```python
from build123d import *

# Parameters (mm, degrees)
SKETCH1_R             = 15
BOSS_EXTRUDE1_DEPTH   = 1075
SKETCH2_R             = 11
BOSS_EXTRUDE2_DEPTH   = 10
BOSS_EXTRUDE3_START   = 10
SKETCH3_R             = 11
BOSS_EXTRUDE3_DEPTH   = 10
M8_TAPPED_HOLE1_D     = 6.8
M8_TAPPED_HOLE1_DEPTH = 19.75
M8_TAPPED_HOLE1_TIP   = 2.042926105
M8_TAPPED_HOLE2_D     = 6.8
M8_TAPPED_HOLE2_DEPTH = 19.75
M8_TAPPED_HOLE2_TIP   = 2.042926105


with BuildPart() as part:
    # Sketch1 → Boss-Extrude1 (new body)
    with BuildSketch(Plane(origin=(0, 0, 0), x_dir=(1, 0, 0), z_dir=(0, 1, 0))):
        with Locations(Location((0, 0, 0), (0, 0, 270))):
            Circle(SKETCH1_R)
    extrude(amount=BOSS_EXTRUDE1_DEPTH)

    # Sketch2 → Boss-Extrude2 (add)
    with BuildSketch(Plane(origin=(0, 1075, 0), x_dir=(1, 0, 0), z_dir=(0, 1, 0))):
        with Locations(Location((0, 0, 0), (0, 0, 270))):
            Circle(SKETCH2_R)
    extrude(amount=BOSS_EXTRUDE2_DEPTH)

    # Sketch3 → Boss-Extrude3 (add)
    with BuildSketch(Plane.XZ.offset(BOSS_EXTRUDE3_START)):
        with Locations(Location((0, 0, 0), (0, 0, 90))):
            Circle(SKETCH3_R)
    extrude(amount=-BOSS_EXTRUDE3_DEPTH)

    # M8 Tapped Hole1
    with Locations(Plane(origin=(0, -10, 0), x_dir=(-1, 0, 0), z_dir=(0, -1, 0))):
        with Locations((0, 0)):
            Hole(M8_TAPPED_HOLE1_D / 2, depth=M8_TAPPED_HOLE1_DEPTH)
            with Locations((0, 0, -(M8_TAPPED_HOLE1_DEPTH + M8_TAPPED_HOLE1_TIP / 2))):  # 118° drill point
                Cone(0, M8_TAPPED_HOLE1_D / 2, M8_TAPPED_HOLE1_TIP, mode=Mode.SUBTRACT)

    # M8 Tapped Hole2
    with Locations(Plane(origin=(0, 1085, 0), x_dir=(1, 0, 0), z_dir=(0, 1, 0))):
        with Locations((0, 0)):
            Hole(M8_TAPPED_HOLE2_D / 2, depth=M8_TAPPED_HOLE2_DEPTH)
            with Locations((0, 0, -(M8_TAPPED_HOLE2_DEPTH + M8_TAPPED_HOLE2_TIP / 2))):  # 118° drill point
                Cone(0, M8_TAPPED_HOLE2_D / 2, M8_TAPPED_HOLE2_TIP, mode=Mode.SUBTRACT)


solid = part.part
```
Build history of the part. All positions in model axes, mm. A direction names the side the tool comes from. Round coordinates to 2 decimals unless told otherwise and drop trailing zeros. Write each loop counter-clockwise with the first axis right and the second up, starting at its lowest first coordinate (ties: lowest second). Pieces come first, ordered by that corner, then holes.
1) Drill centre lines: probe 1 along Y at (x, z) = (0.75, 13); probe 2 along Z at (x, y) = (-0.5, 822); probe 3 along Z at (x, y) = (-2.25, 937). Where is each one in solid material? Low to high.
2) 3-axis set-ups, long thin cutter, end or side, ignore diameter. For faces 1 (the cylindrical face through (-10.74, 1079.93, -2.38)), 2 (the flat face through (10, 0, -5)), 3 (the cylindrical face through (0.66, 529.975, -14.985)): which of +Z, -Z, +X, -X, +Y, -Y reach the whole face in a straight line?
3) Pin check, flat tips, straight feed: pin 1 (6 mm diameter, centred on x = 0, z = 0, fed in from +Y); pin 2 (3 mm diameter, centred on x = 8.5, y = 109, fed in from +Z); pin 3 (8 mm diameter, centred on x = 5, y = 394, fed in from -Z). Stop position of each tip, or through.
4) Band-saw the part on A-A, the plane y = 407. List the corners of the cut face in (x, z).
Ans:
1. probe 1: y = 0 to 1075
1. probe 2: z = -14.99 to 14.99
1. probe 3: z = -14.83 to 14.83
2. face 1: +Y
2. face 2: -Y
2. face 3: +Y, -Y
3. pin 1: stops at y = 1065.01
3. pin 2: stops at z = 13.27
3. pin 3: stops at z = -14.97
4. outline: circle Ø30 at (0, 0)
